Geometry: final body of the model. Coordinates: model frame, mm. A direction names the side the tool comes from. Give positions to 0.01 mm unless a question says otherwise; leave off trailing zeros. Write each loop counter-clockwise with the first axis right and the second up, starting at its lowest first coordinate (ties: lowest second). Pieces come first, ordered by that corner, then holes.
Q1. Pin query (flat end, axial travel): pin 1 Ø16 at (x, z) = (147.5, 39.5) entering from +Y; pin 2 Ø1 at (x, z) = (74, 29) entering from -Y; pin 3 Ø15 at (y, z) = (34.5, 31) entering from -X; pin 4 Ø4 at (x, y) = (36.5, 3.5) entering from -Z. Return the tip coordinate at first contact, or that it passes through.
Q2. Section B-B (x = 147). Return the cut outline in (y, z), plus the area to 3 significant figures.
Q3. Section C-C (y = 33). Return the cut outline in (x, z).
Q4. Line query: line 1 (X direction, y = 10, z = 33.5); line 2 (Y direction, x = 94.5, z = 12.5); line 3 (Y direction, x = 61, z = 16). Output: solid intervals per line, ascending.
Q5. Section D-D (z = 35). Return the cut outline in (x, y), plus the area to 3 significant figures.
Q6. Mould query, pull axis X, two halves, no side actions, for faces 4 (the flat face through (147, 5, 35)), 5 (the flat face through (46, 0, 35)), 6 (the flat face through (80, 30, 30)). Classes: +X half, -X half, draft (parallel to the pull), parting line (faces both ways), or undercut.
Q7. Section A-A (z = 51.5). Return the cut outline in (x, y).
Q8. Reachability of faces 1 (the flat face through (70, -2, 35)), 2 (the flat face through (152.9, 15, 26.7)), 3 (the flat face through (101, 4.319, 35)) from +Z, -Z, +X, -X, +Y, -Y: full face, straight path, thin tool, end or side. Return the list, or none.
from build123d import *

# Parameters (mm, degrees)
STEPPED_BLOCK_BODY_DEPTH = 70
HOLE_A_SKETCH_R          = 10
HOLE_A_DEPTH_20_DEPTH    = 20
HOLE_B_SKETCH_R          = 12
HOLE_B_DEPTH_20_DEPTH    = 20
TRIANGULAR_LUG_DEPTH     = 10
ROUND_BOSS_SKETCH_R      = 10
ROUND_BOSS_10MM_DEPTH    = 10
HOLE_C_SKETCH_R          = 10
HOLE_C_DEPTH_10_DEPTH    = 10


with BuildPart() as part:
    # Stepped Block Profile Sketch → Stepped Block Body (new body)
    with BuildSketch(Plane.XY):
        Polygon((70, 0), (70, -5), (80, 4.319056963), (122, 4.319056963), (132, -5), (132, 0), (172, 0), (172, 15), (122, 15), (122, 45), (80, 45), (80, 15), (10, 15), (10, 0), align=None)
    extrude(amount=STEPPED_BLOCK_BODY_DEPTH)

    # Hole A Sketch → Hole A Depth 20 (cut)
    with BuildSketch(Plane(origin=(0, 15, 0), x_dir=(1, 0, 0), z_dir=(0, 1, 0))):
        with Locations(Location((30, -33.856567252, 0), (0, 0, 270))):
            Circle(HOLE_A_SKETCH_R)
    extrude(amount=-HOLE_A_DEPTH_20_DEPTH, mode=Mode.SUBTRACT)

    # Hole B Sketch → Hole B Depth 20 (cut)
    with BuildSketch(Plane(origin=(0, 45, 0), x_dir=(1, 0, 0), z_dir=(0, 1, 0))):
        with Locations(Location((99.347169036, -33.296354443, 0), (0, 0, 180))):
            Circle(HOLE_B_SKETCH_R)
    extrude(amount=-HOLE_B_DEPTH_20_DEPTH, mode=Mode.SUBTRACT)

    # Triangular Lug Sketch → Triangular Lug (add)
    with BuildSketch(Plane.XY.offset(70)):
        Polygon((10, 15), (80, 15), (80, 45), align=None)
    extrude(amount=-TRIANGULAR_LUG_DEPTH)

    # Round Boss Sketch → Round Boss 10mm (add)
    with BuildSketch(Plane(origin=(0, 15, 0), x_dir=(1, 0, 0), z_dir=(0, 1, 0))):
        with Locations((147.541656159, -38.188385292)):
            Circle(ROUND_BOSS_SKETCH_R)
    extrude(amount=-ROUND_BOSS_10MM_DEPTH)

    # Hole C Sketch → Hole C Depth 10 (cut)
    with BuildSketch(Plane(origin=(0, 15, 0), x_dir=(1, 0, 0), z_dir=(0, 1, 0))):
        with Locations(Location((147, -35, 0), (0, 0, 270))):
            Circle(HOLE_C_SKETCH_R)
    extrude(amount=-HOLE_C_DEPTH_10_DEPTH, mode=Mode.SUBTRACT)


solid = part.part
Computed:
1. pin 1: stops at y = 15
1. pin 2: stops at y = -1.74
1. pin 3: stops at x = 80
1. pin 4: stops at z = 0
2. outline: (0, 0) - (15, 0) - (15, 25) - (5, 25) - (5, 45) - (15, 45) - (15, 70) - (0, 70) - close
2. area: 850 mm2
3. outline: (52, 60) - (80, 60) - (80, 0) - (122, 0) - (122, 70) - (52, 70) - close; hole circle Ø24 at (99.35, 33.3)
4. line 1: x = 10 to 20.01, 39.99 to 137.11, 156.89 to 172
4. line 2: y = 4.32 to 45
4. line 3: y = 0 to 15
5. outline: (10, 0) - (20.07, 0) - (20.07, 15) - (10, 15) - close; (39.93, 0) - (70, 0) - (70, -5) - (80, 4.32) - (122, 4.32) - (132, -5) - (132, 0) - (172, 0) - (172, 15) - (157, 15) - (157, 5) - (137, 5) - (137, 15) - (122, 15) - (122, 45) - (111.23, 45) - (111.23, 25) - (87.47, 25) - (87.47, 45) - (80, 45) - (80, 15) - (39.93, 15) - close
5. area: 2,540 mm2
6. face 4: undercut
6. face 5: draft
6. face 6: -X half
7. outline: (10, 0) - (70, 0) - (70, -5) - (80, 4.32) - (122, 4.32) - (132, -5) - (132, 0) - (172, 0) - (172, 15) - (122, 15) - (122, 45) - (80, 45) - (80, 15) - (10, 15) - close
8. face 1: +Z, -Z, -X, -Y
8. face 2: +Z, -Z, +X, +Y
8. face 3: +Z, -Z, -Y
